```python
from build123d import *

# Parameters (mm, degrees)
SKETCH1_R           = 12.5
SKETCH1_R_2         = 6.25
BOSS_EXTRUDE1_DEPTH = 5


with BuildPart() as part:
    # Sketch1 → Boss-Extrude1 (new body)
    # profile 1 of 2: a face of its own
    with BuildSketch(Plane.XY):
        with BuildLine():
            Line((-24.979991994, 189), (-24.979991994, 1))
            ThreePointArc((-24.979991994, 1), (-3.039752634, 24.814509947), (24, 7))
            Line((24, 7), (-0.810252343, 188.64671282))
            ThreePointArc((-0.810252343, 188.64671282), (0.4895755, 195.089129783), (5.507645346, 199.333333333))
            ThreePointArc((5.507645346, 199.333333333), (-8.535525821, 202.941354129), (-9.722087316, 217.391978417))
            Line((-9.722087316, 217.391978417), (-23.573668252, 194.113582733))
            ThreePointArc((-23.573668252, 194.113582733), (-24.622003262, 191.651719953), (-24.979991994, 189))
        make_face()
    # profile 2 of 2: a face of its own
    with BuildSketch(Plane.XY):
        with Locations((1.020008006, 211)):
            Circle(SKETCH1_R)
        with Locations((1.020008006, 211)):
            Circle(SKETCH1_R_2, mode=Mode.SUBTRACT)
    extrude(amount=BOSS_EXTRUDE1_DEPTH)


solid = part.part
```
Geometry: final body of the model. Coordinates: model frame, mm. Round coordinates to 2 decimals unless told otherwise and drop trailing zeros. Order: outer loops, then holes, each group sorted by start corner. A loop starts at its lowest first (then second) coordinate and runs counter-clockwise, first axis right, second up. Notation, with made-up numbers: M 62,35.5 L 80,35.5 A15 ccw 80,59.5 Z; hole C -23.75,82.25 d3. An arc over 180 degrees is marked long. One line per item, written item: value.
(1) Cut plane A-A (z = 2.55). Return the cut outline in (x, y).
Result sheet:
outline: M -24.98,1 A25 cw 24,7 L -0.81,188.65 A10 cw 5.51,199.33 A12.5 ccw long -9.72,217.39 L -23.57,194.11 A10 ccw -24.98,189 Z; hole C 1.02,211 d12.5
(2) Line query: probe 1 along Y at (x, z) = (-18, 4.4); probe 2 along X at (y, z) = (150, 1.3); probe 3 along Y at (x, z) = (-21, 0.3). Output: solid intervals per line, ascending. Write a range as [from, to].
Result sheet:
probe 1: [17.35, 203.48]
probe 2: [-24.98, 4.47]
probe 3: [13.56, 198.44]
(3) Cut plane B-B (y = 211). Return the cut outline in (x, z), and give its area (3 significant figures).
Result sheet:
outline: M -13.53,0 L -5.23,0 L -5.23,5 L -13.53,5 Z; M 7.27,0 L 13.52,0 L 13.52,5 L 7.27,5 Z
area: 72.7 mm2
(4) Pull-direction query (Y, two-part tool) for faces 1 (the flat face through (-16.55, 205.92, 2.46)), 2 (the flat face through (11.77, 96.55, 2.46)), 3 (the flat face through (-6, 114, 0)); classes: pulls with the +Y half, pulls with the -Y half, needs draft (parallel to the pull), parting line crosses it, or undercut.
Result sheet:
face 1: pulls with the +Y half
face 2: undercut
face 3: needs draft
(5) Cut plane D-D (y = 127). Return the cut outline in (x, z).
Result sheet:
outline: M -24.98,0 L 7.61,0 L 7.61,5 L -24.98,5 Z
(6) Cut plane C-C (x = -16). Return the cut outline in (y, z).
Result sheet:
outline: M 19.21,0 L 206.84,0 L 206.84,5 L 19.21,5 Z
